```python
from build123d import *

# Parameters (mm, degrees)
SKETCH1_W             = 250
SKETCH1_H             = 100
SKETCH1_R             = 2.5
BOSS_EXTRUDE1_DEPTH   = 14
M8_TAPPED_HOLE1_D     = 6.8
M8_TAPPED_HOLE1_DEPTH = 19.75
M8_TAPPED_HOLE1_TIP   = 2.042926105
M8_TAPPED_HOLE2_D     = 6.8


with BuildPart() as part:
    # Sketch1 → Boss-Extrude1 (new body)
    with BuildSketch(Plane.XY):
        with Locations((125, 50)):
            Rectangle(SKETCH1_W, SKETCH1_H)
        with Locations((117, 78)):
            Circle(SKETCH1_R, mode=Mode.SUBTRACT)
        with Locations((173, 78)):
            Circle(SKETCH1_R, mode=Mode.SUBTRACT)
        with Locations((117, 22)):
            Circle(SKETCH1_R, mode=Mode.SUBTRACT)
        with Locations((173, 22)):
            Circle(SKETCH1_R, mode=Mode.SUBTRACT)
    extrude(amount=BOSS_EXTRUDE1_DEPTH)

    # M8 Tapped Hole1
    with Locations(Plane.XY.offset(14)):
        with Locations((117, 78), (173, 78), (117, 22), (173, 22)):
            Hole(M8_TAPPED_HOLE1_D / 2, depth=M8_TAPPED_HOLE1_DEPTH)
            with Locations((0, 0, -(M8_TAPPED_HOLE1_DEPTH + M8_TAPPED_HOLE1_TIP / 2))):  # 118° drill point
                Cone(0, M8_TAPPED_HOLE1_D / 2, M8_TAPPED_HOLE1_TIP, mode=Mode.SUBTRACT)

    # M8 Tapped Hole2 (through all)
    with Locations(Plane.XY.offset(14)):
        with Locations((38, 70), (38, 30)):
            Hole(M8_TAPPED_HOLE2_D / 2)


solid = part.part
```
Geometry: final body of the model. Coordinates: model frame, mm. Coordinates: 2 decimals unless noted, no trailing zeros. Write each loop counter-clockwise with the first axis right and the second up, starting at its lowest first coordinate (ties: lowest second). Pieces come first, ordered by that corner, then holes. Notation, with made-up numbers: M 17,36.5 L 57,36.5 A16 ccw 57,58.5 Z; hole C 54.25,5 d11. An arc over 180 degrees is marked long. Use CSV: the item, a comma, the result in double quotes. Start each with the question number.
1. Cut plane A-A on y = 22. Return the cut outline in (x, z).
2. Cut plane B-B on x = 38. Return the cut outline in (y, z).
3. Mould query, pull axis X, two halves, no side actions, for faces 1 (the face through (123, 51, 14)), 2 (the face through (0, 49, 7)), 3 (the face through (176.4, 22.1, 6.9)), 4 (the face through (119.698, 75.931, 6.902)). Classes: pulls with the +X half, pulls with the -X half, needs draft (parallel to the pull), parting line crosses it, or undercut.
4. First-contact query: P1, Ø6, axis at x = 38, y = 70, coming from the +Z side. Flat tip, straight axial feed; report the tip coordinate or a pass-through.
5. Ray query, probe 1 along Y at (x, z) = (173, 4); probe 2 along Y at (x, z) = (38, 8.5); probe 3 along X at (y, z) = (32.5, 8.5). Return the intervals inside material, ascending.
Entries:
1,outline,"M 0,0 L 113.6,0 L 113.6,14 L 0,14 Z; M 120.4,0 L 169.6,0 L 169.6,14 L 120.4,14 Z; M 176.4,0 L 250,0 L 250,14 L 176.4,14 Z"
2,outline,"M 0,0 L 26.6,0 L 26.6,14 L 0,14 Z; M 33.4,0 L 66.6,0 L 66.6,14 L 33.4,14 Z; M 73.4,0 L 100,0 L 100,14 L 73.4,14 Z"
3,face 1,"needs draft"
3,face 2,"pulls with the -X half"
3,face 3,"undercut"
3,face 4,"undercut"
4,P1,"through"
5,probe 1,"0 to 18.6, 25.4 to 74.6, 81.4 to 100"
5,probe 2,"0 to 26.6, 33.4 to 66.6, 73.4 to 100"
5,probe 3,"0 to 35.7, 40.3 to 250"
